from build123d import *

# Parameters (mm, degrees)
SKETCH_1_R      = 5
EXTRUDE_1_DEPTH = 72.5
SKETCH_2_W      = 590
SKETCH_2_H      = 145
EXTRUDE_2_DEPTH = 1
EXTRUDE_3_DEPTH = 5
SKETCH_5_R      = 5
EXTRUDE_4_DEPTH = 10


with BuildPart() as part:
    # Sketch 1 → Extrude 1 (new, symmetric)
    with BuildSketch(Plane.XY):
        with BuildLine():
            Line((-10, 0), (-10, 10))
            Line((-10, 10), (10, 10))
            Line((10, 10), (10, 0))
            ThreePointArc((10, 0), (0, -10), (-10, 0))
        make_face()
        Circle(SKETCH_1_R, mode=Mode.SUBTRACT)
    extrude(amount=EXTRUDE_1_DEPTH, both=True)



with BuildPart() as body_2:
    # Sketch 2 → Extrude 2 (new body)
    with BuildSketch(Plane(origin=(0, 10, 0), x_dir=(1, 0, 0), z_dir=(0, 1, 0))):
        Rectangle(SKETCH_2_W, SKETCH_2_H)
    extrude(amount=EXTRUDE_2_DEPTH)


with BuildPart() as part_1:
    add(part.part)

    add(body_2.part)  # Extrude 3 merges body 2
    # Sketch 4 → Extrude 3 (add, symmetric)
    with BuildSketch(Plane.XY):
        with BuildLine():
            Line((-10, 10), (-250, 10))
            Line((-250, 10), (-250, 5))
            Line((-250, 5), (-0.599640103, -9.982005397))
            ThreePointArc((-0.599640103, -9.982005397), (-7.279986299, -6.85578584), (-10, 0))
            Line((-10, 0), (-10, 10))
        make_face()
        with BuildLine():
            Line((10, 10), (249.997916658, 11))
            Line((249.997916658, 11), (249.997916658, 6))
            Line((249.997916658, 6), (0.639514993, -9.979530078))
            ThreePointArc((0.639514993, -9.979530078), (7.293666771, -6.84122979), (10, 0))
            Line((10, 0), (10, 10))
        make_face()
    extrude(amount=EXTRUDE_3_DEPTH, both=True)

    # Sketch 5 → Extrude 4 (add)
    with BuildSketch(Plane.XY.offset(72.5)):
        with BuildLine():
            Line((-10, 0), (-10, -10))
            Line((-10, -10), (-5, -10))
            Line((-5, -10), (-5, -25))
            Line((-5, -25), (-5, -35))
            Line((-5, -35), (5, -35))
            Line((5, -35), (5, -25))
            Line((5, -25), (5, -10))
            Line((5, -10), (10, -10))
            Line((10, -10), (10, 0))
            ThreePointArc((10, 0), (0, 10), (-10, 0))
        make_face()
        Circle(SKETCH_5_R, mode=Mode.SUBTRACT)
    extrude(amount=EXTRUDE_4_DEPTH)


solid = part_1.part
Input: part model. Units: mm. Frame: model coordinates. A direction names the side the tool comes from. Give positions to 0.01 mm unless a question says otherwise; leave off trailing zeros. Order: outer loops, then holes, each group sorted by start corner. A loop starts at its lowest first (then second) coordinate and runs counter-clockwise, first axis right, second up. Notation, with made-up numbers: (10, 34) - (43, 34) arc R30 ccw to (43, 68) - close; hole circle Ø10 at (0, -20.5). An arc over 180 degrees is marked (long way). Answer as a JSON object with one key per item and string values. Group by question number.
Q1. Line query: probe 1 along Y at (x, z) = (0, 13); probe 2 along Y at (x, z) = (39, -54.5); probe 3 along Z at (x, y) = (-14.5, 4). Output: solid intervals per line, ascending.
Q2. Mould query, pull axis Y, two halves, no side actions, for faces 1 (the face through (0, 10, 77)), 2 (the face through (-10, 5, 39)), 3 (the face through (-1.08, -4.88, 3.91)), 4 (the face through (127.06, -1.88, 0.07)). Classes: pulls with the +Y half, pulls with the -Y half, needs draft (parallel to the pull), parting line crosses it, or undercut.
Q3. First-contact query: pin 1 Ø3 at (y, z) = (-26.5, 76.5) entering from -X; pin 2 Ø10 at (x, y) = (113.5, -1) entering from +Z; pin 3 Ø1.5 at (x, z) = (-19.5, 47) entering from -Y. Flat tips, straight axial feed; report the tip coordinate or a pass-through.
Q4. Cut plane C-C, the plane y = -21.5. Output: boundary loops of the cut face in (x, z), then the cut area to 3 significant figures.
Q5. Set-up query: faces 5 (the face through (-5, -22, 77)), 6 (the face through (5, -23, 77)), 7 (the face through (-10, 5, -38)), 8 (the face through (10, -5, 77)), 9 (the face through (-10, -5, 77)). Return all of +Z, -Z, +X, -X, +Y, -Y with unobstructed straight access to the full face (end or side cutting, diameter ignored); none if empty.
Q6. Cut plane B-B, the plane x = 119. Output: boundary loops of the cut face in (y, z), then the cut area to 3 significant figures.
Q7. Cut plane A-A, the plane z = -39. Output: boundary loops of the cut face in (x, y), then the cut area to 3 significant figures.
Results:
{
 "1": {"probe 1": "-10 to -5, 5 to 11", "probe 2": "10 to 11", "probe 3": "-5 to 5"},
 "2": {"face 1": "pulls with the +Y half", "face 2": "needs draft", "face 3": "undercut", "face 4": "pulls with the -Y half"},
 "3": {"pin 1": "x = -5", "pin 2": "z = 5", "pin 3": "y = 10"},
 "4": {"outline": "(-5, 72.5) - (5, 72.5) - (5, 82.5) - (-5, 82.5) - close", "area": "100 mm^2"},
 "5": {"face 5": "+Z, -Z, -X, -Y", "face 6": "+Z, -Z, +X, -Y", "face 7": "-Z, -X, -Y", "face 8": "+Z, +X, +Y, -Y", "face 9": "+Z, -X, +Y, -Y"},
 "6": {"outline": "(-2.39, -5) - (10, -5) - (10, -72.5) - (11, -72.5) - (11, 72.5) - (10, 72.5) - (10, 5) - (-2.39, 5) - close", "area": "269 mm^2"},
 "7": {"outline": "(-295, 10) - (-10, 10) - (-10, 0) arc R10 ccw to (10, 0) - (10, 10) - (295, 10) - (295, 11) - (-295, 11) - close; hole circle Ø10 at (0, 0)", "area": "869 mm^2"}
}
